from build123d import *

# Parameters (mm, degrees)
BENT_STRAP_BODY_DEPTH      = 40
SLOTS_3X6_WIDE_REACH       = 118.826
SPLIT_CLAMP_RING_CUT_REACH = 114.485
END_TAB_NOTCH_11X8_REACH   = 108.308
END_TAB_NOTCH_SKETCH_W     = 11
END_TAB_NOTCH_SKETCH_H     = 16


with BuildPart() as part:
    # Strap Profile Sketch → Bent Strap Body (new body)
    with BuildSketch(Plane.XY):
        with BuildLine():
            Line((0, 27), (0, 10))
            ThreePointArc((0, 10), (2.928932188, 2.928932188), (10, 0))
            Line((10, 0), (49.008063966, 0))
            ThreePointArc((49.008063966, 0), (51.911126713, -0.356451285), (54.641722719, -1.404628886))
            Line((54.641722719, -1.404628886), (102, -26.585471583))
            Line((102, -26.585471583), (104.816829377, -21.287786026))
            Line((104.816829377, -21.287786026), (57.458552096, 3.893056671))
            ThreePointArc((57.458552096, 3.893056671), (53.362658087, 5.465323073), (49.008063966, 6))
            Line((49.008063966, 6), (10, 6))
            ThreePointArc((10, 6), (7.171572875, 7.171572875), (6, 10))
            Line((6, 10), (6, 27))
            Line((6, 27), (0, 27))
        make_face()
    extrude(amount=BENT_STRAP_BODY_DEPTH)

    # Slots Sketch → Slots 3x6 Wide (cut, up to next)
    with BuildSketch(Plane(origin=(0, 6, 0), x_dir=(1, 0, 0), z_dir=(0, 1, 0)), mode=Mode.PRIVATE) as slots_3x6_wide_sk1:
        with BuildLine():
            Line((25, -17), (43, -17))
            ThreePointArc((43, -17), (46, -20), (43, -23))
            Line((43, -23), (25, -23))
            ThreePointArc((25, -23), (22, -20), (25, -17))
        make_face()
    slots_3x6_wide_tool1 = extrude(slots_3x6_wide_sk1.sketch, amount=-SLOTS_3X6_WIDE_REACH, mode=Mode.PRIVATE) & part.part
    # Slots Sketch → Slots 3x6 Wide (cut, up to next)
    with BuildSketch(Plane(origin=(0, 6, 0), x_dir=(1, 0, 0), z_dir=(0, 1, 0)), mode=Mode.PRIVATE) as slots_3x6_wide_sk2:
        with BuildLine():
            Line((25, -5), (43, -5))
            ThreePointArc((43, -5), (46, -8), (43, -11))
            Line((43, -11), (25, -11))
            ThreePointArc((25, -11), (22, -8), (25, -5))
        make_face()
    slots_3x6_wide_tool2 = extrude(slots_3x6_wide_sk2.sketch, amount=-SLOTS_3X6_WIDE_REACH, mode=Mode.PRIVATE) & part.part
    # Slots Sketch → Slots 3x6 Wide (cut, up to next)
    with BuildSketch(Plane(origin=(0, 6, 0), x_dir=(1, 0, 0), z_dir=(0, 1, 0)), mode=Mode.PRIVATE) as slots_3x6_wide_sk3:
        with BuildLine():
            Line((25, -29), (43, -29))
            ThreePointArc((43, -29), (46, -32), (43, -35))
            Line((43, -35), (25, -35))
            ThreePointArc((25, -35), (22, -32), (25, -29))
        make_face()
    slots_3x6_wide_tool3 = extrude(slots_3x6_wide_sk3.sketch, amount=-SLOTS_3X6_WIDE_REACH, mode=Mode.PRIVATE) & part.part
    add(slots_3x6_wide_tool1.solids().sort_by_distance((34, 6, 20))[0], mode=Mode.SUBTRACT)
    add(slots_3x6_wide_tool2.solids().sort_by_distance((34, 6, 8))[0], mode=Mode.SUBTRACT)
    add(slots_3x6_wide_tool3.solids().sort_by_distance((34, 6, 32))[0], mode=Mode.SUBTRACT)

    # Split Clamp Ring Sketch → Split Clamp Ring Cut (cut, up to next)
    with BuildSketch(Plane(origin=(14.277813886, 26.852662444, 0), x_dir=(0.8829475928589264, -0.46947156278589186, 0), z_dir=(0.46947156278589186, 0.8829475928589264, 0)), mode=Mode.PRIVATE) as split_clamp_ring_cut_sk1:
        with BuildLine():
            Line((90.978707319, -4.864489093), (85.712943597, -9.605804045))
            ThreePointArc((85.712943597, -9.605804045), (68.244328132, -28.698697883), (89.058596629, -13.321528173))
            Line((89.058596629, -13.321528173), (94.324360351, -8.580213221))
            ThreePointArc((94.324360351, -8.580213221), (95.630838293, -29.262944036), (77.905210863, -40))
            Line((77.905210863, -40), (102.541777363, -40))
            Line((102.541777363, -40), (102.541777363, 0))
            Line((102.541777363, 0), (77.905210863, 0))
            ThreePointArc((77.905210863, 0), (84.879799807, -1.255531241), (90.978707319, -4.864489093))
        make_face()
    split_clamp_ring_cut_tool1 = extrude(split_clamp_ring_cut_sk1.sketch, amount=-SPLIT_CLAMP_RING_CUT_REACH, mode=Mode.PRIVATE) & part.part
    add(split_clamp_ring_cut_tool1.solids().sort_by_distance((89.983505, -13.400768, 19.581438))[0], mode=Mode.SUBTRACT)

    # End Tab Notch Sketch → End Tab Notch 11x8 (cut, up to next)
    with BuildSketch(Plane(origin=(6, 0, 0), x_dir=(0, 0, -1), z_dir=(1, 0, 0)), mode=Mode.PRIVATE) as end_tab_notch_11x8_sk1:
        with Locations((-20, 27)):
            Rectangle(END_TAB_NOTCH_SKETCH_W, END_TAB_NOTCH_SKETCH_H)
    end_tab_notch_11x8_tool1 = extrude(end_tab_notch_11x8_sk1.sketch, amount=-END_TAB_NOTCH_11X8_REACH, mode=Mode.PRIVATE) & part.part
    add(end_tab_notch_11x8_tool1.solids().sort_by_distance((6, 27, 20))[0], mode=Mode.SUBTRACT)


solid = part.part
Geometry: final body of the model. Coordinates: model frame, mm. A direction names the side the tool comes from. Give positions to 0.01 mm unless a question says otherwise; leave off trailing zeros. Order: outer loops, then holes, each group sorted by start corner. A loop starts at its lowest first (then second) coordinate and runs counter-clockwise, first axis right, second up. Notation, with made-up numbers: (81, -4.5) -> (134, -4.5) arc R29 ccw to (134, 19.5) -> close; hole circle Ø8 at (65, 10). An arc over 180 degrees is marked (long way). Write each question's results on one line, items separated by ' | '.
1) Cut plane A-A (x = 28). Output: boundary loops of the cut face in (y, z).
Geometry says:
outline: (0, 0) -> (6, 0) -> (6, 5) -> (0, 5) -> close; (0, 11) -> (6, 11) -> (6, 17) -> (0, 17) -> close; (0, 23) -> (6, 23) -> (6, 29) -> (0, 29) -> close; (0, 35) -> (6, 35) -> (6, 40) -> (0, 40) -> close
2) Draft query along X for faces 6 (the face through (22, 3, 20)), 7 (the face through (0, 18.6, 19.7)), 8 (the face through (3, 19, 20)). Return one class per face: released by +X, released by -X, zero draft, split by the parting line, or undercut.
Geometry says:
face 6: undercut | face 7: released by -X | face 8: zero draft
3) Set-up query: faces 1 (the face through (35, 5, 0)), 2 (the face through (46, 3, 8)), 3 (the face through (30, 6, 24)), 4 (the face through (97.45, -20.72, 28.99)), 5 (the face through (3, 23, 25.5)). Return all of +Z, -Z, +X, -X, +Y, -Y with unobstructed straight access to the full face (end or side cutting, diameter ignored); none if empty.
Geometry says:
face 1: -Z, +X, -X, +Y, -Y | face 2: +Y, -Y | face 3: +Z, -Z, +X, +Y | face 4: +X, -Y | face 5: +X, -X, +Y
4) Cut plane D-D (y = 11.5). Output: boundary loops of the cut face in (x, z).
Geometry says:
outline: (0, 0) -> (6, 0) -> (6, 40) -> (0, 40) -> close
5) Line query: line 1 along X through (y, z) = (20, 27); line 2 along Z through (x, y) = (88, -16.5). Output: solid intervals per line, ascending.
Geometry says:
line 1: x = 0 to 6 | line 2: z = 1.48 to 9.41, 30.59 to 38.52
6) First-contact query: pin 1 Ø10 at (x, z) = (58.5, 24.5) entering from -Y; pin 2 Ø19.5 at (x, z) = (22, 30) entering from -Y; pin 3 Ø5 at (y, z) = (6, 15) entering from +X; pin 4 Ø1.8 at (x, y) = (2, 22.5) entering from -Z. Flat tips, straight axial feed; report the tip coordinate or a pass-through.
Geometry says:
pin 1: stops at y = -6.11 | pin 2: stops at y = 0 | pin 3: stops at x = 58.2 | pin 4: stops at z = 0
7) Cut plane C-C (z = 20). Output: boundary loops of the cut face in (x, y), and give its area (3 significant figures).
Geometry says:
outline: (0, 10) arc R10 ccw to (10, 0) -> (22, 0) -> (22, 6) -> (10, 6) arc R4 cw to (6, 10) -> (6, 19) -> (0, 19) -> close; (46, 0) -> (49.01, 0) arc R12 cw to (54.64, -1.4) -> (68.77, -8.92) -> (71.59, -3.62) -> (57.46, 3.89) arc R18 ccw to (49.01, 6) -> (46, 6) -> close; (91.73, -21.12) -> (97.91, -24.41) -> (100.72, -19.11) -> (94.54, -15.82) -> close | area: 392 mm²
8) Cut plane B-B (z = 27.5). Output: boundary loops of the cut face in (x, y).
Geometry says:
outline: (0, 10) arc R10 ccw to (10, 0) -> (49.01, 0) arc R12 cw to (54.64, -1.4) -> (70.87, -10.03) -> (73.69, -4.74) -> (57.46, 3.89) arc R18 ccw to (49.01, 6) -> (10, 6) arc R4 cw to (6, 10) -> (6, 27) -> (0, 27) -> close; (89.62, -20) -> (96.62, -23.72) -> (99.43, -18.43) -> (92.44, -14.71) -> close
